The model under review builds one solid part; all positions refer to its coordinate system, in mm. A direction names the side the tool comes from. Give positions to 0.01 mm unless a question says otherwise; leave off trailing zeros. Order: outer loops, then holes, each group sorted by start corner. A loop starts at its lowest first (then second) coordinate and runs counter-clockwise, first axis right, second up. Notation, with made-up numbers: (21.25, 63) - (54.25, 63) arc R10 ccw to (54.25, 77) - close; hole circle Ø7 at (-6.75, 64). An arc over 180 degrees is marked (long way). Use a Markdown table: item, result. Add a question column.
```python
from build123d import *

# Parameters (mm, degrees)
SKETCH_1_R          = 37.5
SKETCH_1_R_2        = 7.5
EXTRUDE_1_DEPTH     = 50
SKETCH_7_W          = 5
SKETCH_7_H          = 4.6
CUT_EXTRUDE_1_DEPTH = 90


with BuildPart() as part:
    # 草图1 → 凸台-拉伸1 (new body)
    with BuildSketch(Plane.XY):
        Circle(SKETCH_1_R)
        Circle(SKETCH_1_R_2, mode=Mode.SUBTRACT)
    extrude(amount=EXTRUDE_1_DEPTH)

    # 草图2 → 切除-旋转1 (revolve, cut)
    with BuildSketch(Plane(origin=(0, 0, 0), x_dir=(1, 0, 0), z_dir=(0, 1, 0))):
        Polygon((-38.25, -17.648818614), (-23.25, -21.25), (-23.25, -28.75), (-38.25, -32.351181386), align=None)
    revolve(axis=Axis((0, 0, 0), (0, 0, 1)), mode=Mode.SUBTRACT)

    # 草图3 → M5 螺纹孔2 (revolve, cut)
    with BuildSketch(Plane(origin=(0, 32.5, 9), x_dir=(0, 0, 1), z_dir=(1, 0, 0))):
        Polygon((0, 0), (0, 31.2618073), (2.1, 30), (2.1, 0), align=None)
    revolve(axis=Axis((0, 38.85, 9), (0, -1, 0)), mode=Mode.SUBTRACT)

    # 草图5 → M5 螺纹孔1 (revolve, cut)
    with BuildSketch(Plane(origin=(32.5, 0, 9), x_dir=(0, 0, -1), z_dir=(0, 1, 0))):
        Polygon((0, 0), (0, 31.2618073), (2.1, 30), (2.1, 0), align=None)
    revolve(axis=Axis((38.85, 0, 9), (-1, 0, 0)), mode=Mode.SUBTRACT)

    # 草图7 → 切除-拉伸1 (cut)
    with BuildSketch(Plane(origin=(0, 0, 0), x_dir=(-1, 0, 0), z_dir=(0, 0, -1))):
        with Locations((0, 7.5)):
            Rectangle(SKETCH_7_W, SKETCH_7_H)
    extrude(amount=-CUT_EXTRUDE_1_DEPTH, mode=Mode.SUBTRACT)


solid = part.part
```
Q1. Draft analysis for pull direction Y (two halves, no side actions). For faces 1 (the flat face through (32.5, 0, 9)), 2 (the conical face through (17.793, -16.316, 28.964)), 3 (the flat face through (-1, -8, 50)), state which applies: pulls with the +Y half, pulls with the -Y half, needs draft (parallel to the pull), parting line crosses it, or undercut.
Q2. Clearance check with flat-ended pins moving along their axes: P1, Ø1, axis at y = 16.5, z = 15.5, coming from the -X side; P2, Ø2, axis at x = 12.5, z = 25.5, coming from the +Y side; P3, Ø1.5, axis at x = -0.5, z = 27, coming from the -Y side. State where each tip first meets the part, or that it passes through.
Q3. We need section D-D (y = 28). Count the separate pieces of the cut face and the enclosed holes in it, plus the area to 3 significant figures.
Q4. We need section A-A (x = 0). Write out the cut boundary in (y, z).
Q5. Wall thickness on probe 1 along Z at (x, y) = (23, 0); probe 2 along X at (y, z) = (0, 13); probe 3 along Z at (x, y) = (0, 27): over which ranges is each line inside the solid? List them lowest first.
Q6. Machinability: for faces 4 (the flat face through (-1, -8, 0)), 5 (the flat face through (2.5, 8, 25)), 6 (the conical face through (18.999, 14.568, 21.084)), which of the approach directions +Z, -Z, +X, -X, +Y, -Y give a long, thin tool a straight path to every point of the face, cutting with its end or side? Answer none if there is none.
Q7. We need section B-B (y = 0). Write out the cut boundary in (x, z).
Q8. We need section C-C (z = 47). Write out the cut boundary in (x, y).
Here are the results:
| question | item | result |
|---|---|---|
| 1 | face 1 | undercut |
| 1 | face 2 | parting line crosses it |
| 1 | face 3 | needs draft |
| 2 | P1 | x = -33.92 |
| 2 | P2 | y = 20.21 |
| 2 | P3 | y = -23.25 |
| 3 | separate pieces | 2 |
| 3 | enclosed holes | 1 |
| 3 | area | 1,910 mm2 |
| 4 | outline | (-37.5, 0) - (-7.5, 0) - (-7.5, 50) - (-37.5, 50) - (-37.5, 32.17) - (-23.25, 28.75) - (-23.25, 21.25) - (-37.5, 17.83) - close; (9.8, 0) - (37.5, 0) - (37.5, 17.83) - (23.25, 21.25) - (23.25, 28.75) - (37.5, 32.17) - (37.5, 50) - (9.8, 50) - (9.8, 11.1) - (32.5, 11.1) - (32.5, 6.9) - (9.8, 6.9) - close |
| 5 | probe 1 | 0 to 6.9, 11.1 to 50 |
| 5 | probe 2 | -37.5 to -7.5, 7.5 to 37.5 |
| 5 | probe 3 | 0 to 6.9, 11.1 to 20.35, 29.65 to 50 |
| 6 | face 4 | -Z, +X, -X, +Y, -Y |
| 6 | face 5 | +Z, -Z |
| 6 | face 6 | none |
| 7 | outline | (-37.5, 0) - (-7.5, 0) - (-7.5, 50) - (-37.5, 50) - (-37.5, 32.17) - (-23.25, 28.75) - (-23.25, 21.25) - (-37.5, 17.83) - close; (7.5, 0) - (37.5, 0) - (37.5, 17.83) - (23.25, 21.25) - (23.25, 28.75) - (37.5, 32.17) - (37.5, 50) - (7.5, 50) - (7.5, 11.1) - (32.5, 11.1) - (32.5, 6.9) - (7.5, 6.9) - close |
| 8 | outline | circle Ø75 at (0, 0); hole (-2.5, 7.07) arc R7.5 ccw (long way) to (2.5, 7.07) - (2.5, 9.8) - (-2.5, 9.8) - close |
